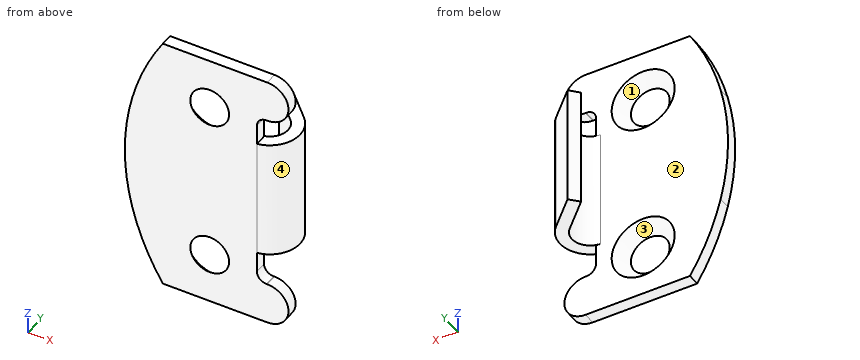
```python
from build123d import *

# Parameters (mm, degrees)
EXTRUDE_1_DEPTH      = 5
EXTRUDE_1_DEPTH_BACK = 5
EXTRUDE_2_DEPTH      = 1
SKETCH_3_W           = 100
SKETCH_3_H           = 100
SKETCH_3_R           = 20.87
CUT_EXTRUDE_1_DEPTH  = 2


with BuildPart() as part:
    # 草图1 → 凸台-拉伸1 (new, two sides: drawn at the far end of the back side and taken through both)
    with BuildSketch(Plane.XY.offset(-EXTRUDE_1_DEPTH_BACK)):
        with BuildLine():
            Line((0, 0), (10.5, 0))
            ThreePointArc((10.5, 0), (12.813469706, 1.552446351), (12.253709329, 4.281713666))
            Line((12.253709329, 4.281713666), (10, 6.5))
            Line((10, 6.5), (9.298516268, 5.787314534))
            Line((9.298516268, 5.787314534), (11.552225598, 3.5690282))
            ThreePointArc((11.552225598, 3.5690282), (11.888081824, 1.931467811), (10.5, 1))
            Line((10.5, 1), (0, 1))
            Line((0, 1), (0, 0))
        make_face()
    extrude(amount=EXTRUDE_1_DEPTH + EXTRUDE_1_DEPTH_BACK)

    # 草图2 → 凸台-拉伸2 (add)
    with BuildSketch(Plane(origin=(0, 0, 0), x_dir=(1, 0, 0), z_dir=(0, 1, 0))):
        with BuildLine():
            Line((3.134247972, -11), (11.75, -11))
            ThreePointArc((11.75, -11), (13.5, -9.25), (11.75, -7.5))
            Line((11.75, -7.5), (11.69, -7.5))
            ThreePointArc((11.69, -7.5), (11.124314575, -7.265685425), (10.89, -6.7))
            Line((10.89, -6.7), (10.89, 6.7))
            ThreePointArc((10.89, 6.7), (11.124314575, 7.265685425), (11.69, 7.5))
            Line((11.69, 7.5), (11.75, 7.5))
            ThreePointArc((11.75, 7.5), (13.5, 9.25), (11.75, 11))
            Line((11.75, 11), (3.134247972, 11))
            ThreePointArc((3.134247972, 11), (0, 0), (3.134247972, -11))
        make_face()
    extrude(amount=EXTRUDE_2_DEPTH)

    # 草图3 → 切除-拉伸1 (cut)
    with BuildSketch(Plane(origin=(0, 0, 0), x_dir=(1, 0, 0), z_dir=(0, 1, 0))):
        Rectangle(SKETCH_3_W, SKETCH_3_H)
        with Locations((20.87, 0)):
            Circle(SKETCH_3_R, mode=Mode.SUBTRACT)
    extrude(amount=CUT_EXTRUDE_1_DEPTH, mode=Mode.SUBTRACT)

    # 草图4 → 切除-旋转1 (revolve, cut)
    with BuildSketch(Plane.XY.offset(6.75), mode=Mode.PRIVATE) as cut_revolve_1_sk:
        Polygon((7, 1), (9.6, 1), (8.6, 0), (7, 0), align=None)
    revolve(cut_revolve_1_sk.sketch.rotate(Axis((7, 0, 6.75), (0, 1, 0)), 270), axis=Axis((7, 0, 6.75), (0, 1, 0)), mode=Mode.SUBTRACT)

    # 草图5 → 切除-旋转2 (revolve, cut)
    with BuildSketch(Plane.XY.offset(-6.75), mode=Mode.PRIVATE) as cut_revolve_2_sk:
        Polygon((7, 1), (9.6, 1), (8.6, 0), (7, 0), align=None)
    revolve(cut_revolve_2_sk.sketch.rotate(Axis((7, 0, -6.75), (0, 1, 0)), 270), axis=Axis((7, 0, -6.75), (0, 1, 0)), mode=Mode.SUBTRACT)


solid = part.part
```
Work out the finished part from the listing and answer in its coordinate system (mm). Face numbers are marked on the shaded views. A direction names the side the tool comes from. Round coordinates to 2 decimals unless told otherwise and drop trailing zeros. Write each loop counter-clockwise with the first axis right and the second up, starting at its lowest first coordinate (ties: lowest second). Pieces come first, ordered by that corner, then holes. Notation, with made-up numbers: (47.5, 27.5) -> (98.5, 27.5) arc R17 ccw to (98.5, 42.5) -> close; hole circle Ø4 at (-35.5, -12). An arc over 180 degrees is marked (long way). Write each question's results on one line, items separated by ' | '.
Q1. Straight lines are drawn through the part: line 1 along Z through (x, y) = (8.25, 0.75); line 2 along Y through (x, z) = (1.5, -3.25); line 3 along X through (y, z) = (6, 4.75). For each, find the intervals that lie inside material, in ascending order. Write a range as [from, to].
Data:
line 1: [-11, -8.74], [-4.76, 4.76], [8.74, 11] | line 2: [0, 1] | line 3: [9.51, 10.51]
Q2. Section A-A, the plane x = 7 is taken. Write down the section's boundary in (y, z), then the cut area to 3 significant figures.
Data:
outline: (0, -11) -> (1, -11) -> (1, -9.35) -> (0, -8.35) -> close; (0, -5.15) -> (1, -4.15) -> (1, 4.15) -> (0, 5.15) -> close; (0, 8.35) -> (1, 9.35) -> (1, 11) -> (0, 11) -> close | area: 13.6 mm^2
Q3. Flat-ended cylindrical pins translate along their axes: P1, Ø1.1, axis at x = 11, y = 3.5, coming from the -Z side; P2, Ø0.8, axis at y = 0.5, z = 0.5, coming from the +X side. Find the tip coordinate at first contact, or state that the pin passes through.
Data:
P1: z = -5 | P2: x = 12.42
Q4. Section C-C, the plane y = 2.25 is taken. Write down the section's boundary in (x, z).
Data:
outline: (11.98, -5) -> (12.99, -5) -> (12.99, 5) -> (11.98, 5) -> close
Q5. Determine the mould class of the marked faces 1 and 2 for opening direction Z: released by +Z, released by -Z, zero draft, split by the parting line, or undercut.
Data:
face 1: undercut | face 2: zero draft
Q6. Which of the six approach directions +Z, -Z, +X, -X, +Y, -Y give full straight-line access (tool end or side, diameter ignored) to the marked faces 3 and 4?
Data:
face 3: +Y | face 4: +X
